```python
from build123d import *

# Parameters (mm, degrees)
SKETCH_1_W          = 440
SKETCH_1_H          = 436
EXTRUDE_1_DEPTH     = 3
SKETCH_2_W          = 30
SKETCH_2_H          = 30
CUT_EXTRUDE_1_DEPTH = 10
CUT_EXTRUDE_2_DEPTH = 10
CUT_EXTRUDE_3_DEPTH = 10
EXTRUDE_2_DEPTH     = 3
FILLET_1_R          = 5
CUT_EXTRUDE_4_DEPTH = 10


with BuildPart() as part:
    # 草图1 → 凸台-拉伸1 (new body)
    with BuildSketch(Plane.XY):
        Rectangle(SKETCH_1_W, SKETCH_1_H)
    extrude(amount=EXTRUDE_1_DEPTH)

    # 草图2 → 切除-拉伸1 (cut)
    with BuildSketch(Plane.XY.offset(3)):
        with Locations((-205, -203)):
            Rectangle(SKETCH_2_W, SKETCH_2_H)
        with Locations((-205, 203)):
            Rectangle(SKETCH_2_W, SKETCH_2_H)
    extrude(amount=-CUT_EXTRUDE_1_DEPTH, mode=Mode.SUBTRACT)

    # 草图3 → 切除-拉伸2 (cut)
    with BuildSketch(Plane.XY.offset(3)):
        Polygon((220, 218), (20, 218), (220, 18), align=None)
        Polygon((220, -218), (220, -18), (20, -218), align=None)
    extrude(amount=-CUT_EXTRUDE_2_DEPTH, mode=Mode.SUBTRACT)

    # 草图4 → 切除-拉伸3 (cut)
    with BuildSketch(Plane.XY.offset(3)):
        Polygon((220, 18), (184, 54), (184, -54), (220, -18), align=None)
    extrude(amount=-CUT_EXTRUDE_3_DEPTH, mode=Mode.SUBTRACT)

    # 草图5 → 凸台-拉伸2 (add)
    with BuildSketch(Plane.XY.offset(3)):
        Polygon((20, 218), (83.639610307, 154.360389693), (147.279220614, 218), align=None)
        Polygon((152.180194847, 85.819805153), (184, 54), (184, 117.639610307), align=None)
    extrude_2 = extrude(amount=-EXTRUDE_2_DEPTH)

    # 镜向1: 凸台-拉伸2 across plane
    add(extrude_2.mirror(Plane.ZX))

    # 圆角1
    fillet_1_edges = [part.edges().sort_by_distance(p)[0] for p in [
        (83.639610307, 154.360389693, 1.5),
        (147.279220614, 218, 1.5),
        (184, 117.639610307, 1.5),
        (152.180194847, 85.819805153, 1.5),
        (147.279220614, -218, 1.5),
        (184, -117.639610307, 1.5),
    ]]
    fillet(fillet_1_edges, radius=FILLET_1_R)

    # 草图6 → 切除-拉伸4 (cut)
    with BuildSketch(Plane(origin=(0, 0, 0), x_dir=(-1, 0, 0), z_dir=(0, 0, -1))):
        with BuildLine():
            Line((-93, 208.3), (-87, 208.3))
            ThreePointArc((-87, 208.3), (-83.7, 205), (-87, 201.7))
            Line((-87, 201.7), (-93, 201.7))
            ThreePointArc((-93, 201.7), (-96.3, 205), (-93, 208.3))
        make_face()
        with BuildLine():
            Line((87, 208.3), (93, 208.3))
            ThreePointArc((93, 208.3), (96.3, 205), (93, 201.7))
            Line((93, 201.7), (87, 201.7))
            ThreePointArc((87, 201.7), (83.7, 205), (87, 208.3))
        make_face()
        with BuildLine():
            Line((210.3, 123), (210.3, 117))
            ThreePointArc((210.3, 117), (207, 113.7), (203.7, 117))
            Line((203.7, 117), (203.7, 123))
            ThreePointArc((203.7, 123), (207, 126.3), (210.3, 123))
        make_face()
        with BuildLine():
            Line((210.3, -117), (210.3, -123))
            ThreePointArc((210.3, -123), (207, -126.3), (203.7, -123))
            Line((203.7, -123), (203.7, -117))
            ThreePointArc((203.7, -117), (207, -113.7), (210.3, -117))
        make_face()
        with BuildLine():
            Line((93, -208.3), (87, -208.3))
            ThreePointArc((87, -208.3), (83.7, -205), (87, -201.7))
            Line((87, -201.7), (93, -201.7))
            ThreePointArc((93, -201.7), (96.3, -205), (93, -208.3))
        make_face()
        with BuildLine():
            Line((-93, -201.7), (-87, -201.7))
            ThreePointArc((-87, -201.7), (-83.7, -205), (-87, -208.3))
            Line((-87, -208.3), (-93, -208.3))
            ThreePointArc((-93, -208.3), (-96.3, -205), (-93, -201.7))
        make_face()
    extrude(amount=-CUT_EXTRUDE_4_DEPTH, mode=Mode.SUBTRACT)


solid = part.part
```
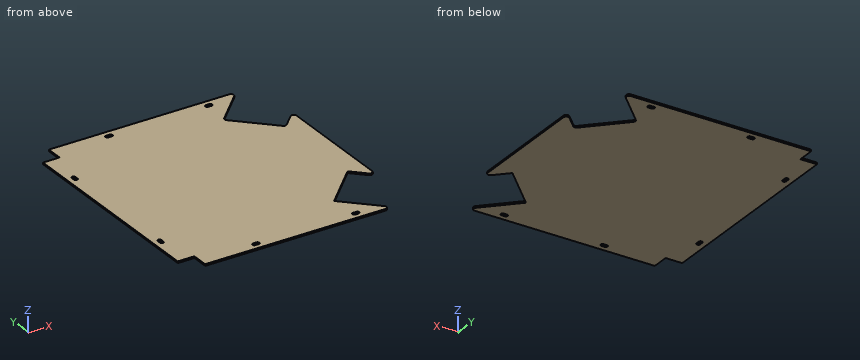
For this review, take the finished solid that the model builds, in its own axes (mm). Give positions to 0.01 mm unless a question says otherwise; leave off trailing zeros. Write each loop counter-clockwise with the first axis right and the second up, starting at its lowest first coordinate (ties: lowest second). Pieces come first, ordered by that corner, then holes.
Item 1: Wall thickness on probe 1 along Y at (x, z) = (123, 1.3); probe 2 along Y at (x, z) = (125, 0.45); probe 3 along X at (y, z) = (194, 0.65): over which ranges is each line inside the solid? List them lowest first.
Item 2: Insertion check: P1, Ø1.5, axis at y = -119, z = 1.5, coming from the +X side; P2, Ø1.5, axis at x = -209.5, z = 1.5, coming from the +Y side. Each pin has a flat end and moves straight along its axis. Give the tip position at first contact, or say it passes through.
Item 3: Take a section at A-A (x = 114.5). Give the boundary of the cut face in (y, z).
Item 4: Take a section at B-B (z = 2.1). Give the number of separate pieces and of enclosed holes in the cut face, and give its area (3 significant figures).
Established:
1. probe 1: y = -218 to -193.72, -115 to 115, 193.72 to 218
1. probe 2: y = -218 to -195.72, -113 to 113, 195.72 to 218
1. probe 3: x = -190 to 123.28
2. P1: stops at x = 119.75
2. P2: stops at y = 188
3. outline: (-218, 0) - (-185.22, 0) - (-185.22, 3) - (-218, 3) - close; (-123.5, 0) - (123.5, 0) - (123.5, 3) - (-123.5, 3) - close; (185.22, 0) - (218, 0) - (218, 3) - (185.22, 3) - close
4. separate pieces: 1
4. enclosed holes: 6
4. area: 157,000 mm2
